```python
from build123d import *

# Parameters (mm, degrees)
BASE_DEPTH          = 2700
FILLET1_R           = 10
FILLET2_R           = 5
SKETCH_1_W          = 118
SKETCH_1_H          = 250
BOSS_EXTRUDE1_DEPTH = 5
SKETCH2_W           = 170
SKETCH2_H           = 262
BOSS_EXTRUDE2_DEPTH = 5
SKETCH3_R           = 50
BOSS_EXTRUDE3_DEPTH = 28


with BuildPart() as part:
    # Sketch1 → Base (new body)
    with BuildSketch(Plane(origin=(0, 0, 0), x_dir=(0, 0, -1), z_dir=(1, 0, 0))):
        Polygon((-59, 0), (59, 0), (59, 7.666666667), (5, 16.666666667), (5, 233.333333333), (59, 242.333333333), (59, 250), (-59, 250), (-59, 242.333333333), (-5, 233.333333333), (-5, 16.666666667), (-59, 7.666666667), align=None)
    extrude(amount=BASE_DEPTH)

    # Fillet1
    fillet1_edges = [part.edges().sort_by_distance(p)[0] for p in [
        (1350, 16.666666667, 5),
        (1350, 233.333333333, 5),
        (1350, 233.333333333, -5),
        (1350, 16.666666667, -5),
    ]]
    fillet(fillet1_edges, radius=FILLET1_R)

    # Fillet2
    fillet2_edges = [part.edges().sort_by_distance(p)[0] for p in [
        (1350, 7.666666667, 59),
        (1350, 242.333333333, 59),
        (1350, 242.333333333, -59),
        (1350, 7.666666667, -59),
    ]]
    fillet(fillet2_edges, radius=FILLET2_R)

    # 草图1 → Boss-Extrude1 (add, symmetric)
    with BuildSketch(Plane.ZY):
        with Locations((0, 125)):
            Rectangle(SKETCH_1_W, SKETCH_1_H)
    extrude(amount=BOSS_EXTRUDE1_DEPTH, both=True)

    # Sketch2 → Boss-Extrude2 (add, symmetric)
    with BuildSketch(Plane(origin=(2700, 0, 0), x_dir=(0, 0, -1), z_dir=(1, 0, 0))):
        with Locations((0, 125)):
            Rectangle(SKETCH2_W, SKETCH2_H)
    extrude(amount=BOSS_EXTRUDE2_DEPTH, both=True)

    # Sketch3 → Boss-Extrude3 (add)
    with BuildSketch(Plane(origin=(0, 0, 0), x_dir=(-1, 0, 0), z_dir=(0, -1, 0))):
        with Locations(Location((-205, 0, 0), (0, 0, 270))):
            Circle(SKETCH3_R)
    extrude(amount=BOSS_EXTRUDE3_DEPTH)


solid = part.part
```
Verification items for the finished model (mm, model axes). A direction names the side the tool comes from. Round coordinates to 2 decimals unless told otherwise and drop trailing zeros. Write each loop counter-clockwise with the first axis right and the second up, starting at its lowest first coordinate (ties: lowest second). Pieces come first, ordered by that corner, then holes. Notation, with made-up numbers: (54.5, -5) -> (62.5, -5) arc R13 ccw to (62.5, 3) -> close; hole circle Ø7 at (58.25, 82.25). An arc over 180 degrees is marked (long way). Write each question's results on one line, items separated by ' | '. Start each with the question number.
1. Cross-section at A-A (x = 1838). Enter the section's corners in (y, z).
2. Draft check along Y on faces 1 (the flat face through (1331, 124, -5)), 2 (the flat face through (1326, 250, -1)), 3 (the flat face through (5, 127, -32)), 4 (the flat face through (-5, 127, -1)). Enter one of: +Y half, -Y half, draft (parallel to the pull), parting line (faces both ways), or undercut.
3. Cross-section at B-B (y = 165.5). Enter the section's corners in (x, z), then the cut area to 3 significant figures.
4. Depth check by flat-ended pin: P1, Ø1, axis at x = 1417.5, z = 18.5, coming from the -Y side; P2, Ø11, axis at x = 2699.5, z = 33, coming from the -Y side; P3, Ø3, axis at x = 879, y = 112.5, coming from the +Z side. Enter the tip coordinate at first touch or a pass-through.
5. Material ranges on probe 1 along X at (y, z) = (214.5, -55.5); probe 2 along X at (y, z) = (151, 70.5); probe 3 along Y at (x, z) = (1157.5, 52), recorded low to high. Write a range as from..to.
6. Set-up check for faces 5 (the cylindrical face through (253.81, -13.8, -10.84)), 6 (the flat face through (1331.17, 238.23, 34.38)), 7 (the flat face through (2695, 127, 20)), 8 (the flat face through (1331.17, 11.77, -34.38)), 9 (the flat face through (204, -28, -1)): record each of +Z, -Z, +X, -X, +Y, -Y from which the full face is reachable in a straight line by a thin tool's end or side.
7. Cross-section at C-C (x = 205). Enter the section's corners in (y, z), then the cut area to 3 significant figures.
Solutions:
1) outline: (0, -59) -> (3.43, -59) arc R5 ccw to (8.36, -54.82) -> (15.27, -13.36) arc R10 cw to (25.14, -5) -> (224.86, -5) arc R10 cw to (234.73, -13.36) -> (241.64, -54.82) arc R5 ccw to (246.57, -59) -> (250, -59) -> (250, 59) -> (246.57, 59) arc R5 ccw to (241.64, 54.82) -> (234.73, 13.36) arc R10 cw to (224.86, 5) -> (25.14, 5) arc R10 cw to (15.27, 13.36) -> (8.36, 54.82) arc R5 ccw to (3.43, 59) -> (0, 59) -> close
2) face 1: undercut | face 2: +Y half | face 3: undercut | face 4: draft
3) outline: (-5, -59) -> (5, -59) -> (5, -5) -> (2695, -5) -> (2695, -85) -> (2705, -85) -> (2705, 85) -> (2695, 85) -> (2695, 5) -> (5, 5) -> (5, 59) -> (-5, 59) -> close | area: 29,800 mm2
4) P1: stops at y = 0 | P2: stops at y = -6 | P3: stops at z = 5
5) probe 1: x = -5..5, 2695..2705 | probe 2: x = 2695..2705 | probe 3: y = 0..8.83, 241.17..250
6) face 5: -Y | face 6: +Z | face 7: none | face 8: -Z | face 9: +Z, -Z, +X, -X, -Y
7) outline: (-28, -50) -> (0, -50) -> (0, -59) -> (3.43, -59) arc R5 ccw to (8.36, -54.82) -> (15.27, -13.36) arc R10 cw to (25.14, -5) -> (224.86, -5) arc R10 cw to (234.73, -13.36) -> (241.64, -54.82) arc R5 ccw to (246.57, -59) -> (250, -59) -> (250, 59) -> (246.57, 59) arc R5 ccw to (241.64, 54.82) -> (234.73, 13.36) arc R10 cw to (224.86, 5) -> (25.14, 5) arc R10 cw to (15.27, 13.36) -> (8.36, 54.82) arc R5 ccw to (3.43, 59) -> (0, 59) -> (0, 50) -> (-28, 50) -> close | area: 7,970 mm2
